The drawing under review shows one solid part. Ordinate dimensions are in mm from its lowest x, y, z. A direction names the side the tool comes from. Coordinates: 2 decimals unless noted, no trailing zeros. Loops run counter-clockwise (first coordinate to the right, second up) from the corner with the lowest first, then second, coordinate; pieces in that order, holes last. Notation, with made-up numbers: (40.5, -11) - (46.5, -11) arc R14 cw to (46.5, 6) - close; hole circle Ø7 at (77.25, 79.25). An arc over 180 degrees is marked (long way). Answer as a JSON object with one key per item and string values. Group by question number.
Item 1: We need section A-A (z = 3.5). Give the boundary of the cut face in (x, y).
Item 2: Clearance check with a flat-ended pin moving along its axis: pin 1 (1.5 mm diameter, centred on y = 3.5, z = 3, fed in from -X). State where the tip first meets the part, or that it passes through.
Item 3: We need section D-D (z = 6.25). Give the boundary of the cut face in (x, y).
Item 4: To check wall thickness, follow line 1 (X direction, y = 1.65, z = 3.5); line 2 (X direction, y = 2.3, z = 4.25); line 3 (Z direction, x = 24.5, y = 2.15). State the ranges of each line that lie inside material, in increasing order.
Item 5: Mouldability with a two-part tool opening along Z and no side actions: class the marked faces 3, 4 and 5 as released by +Z, released by -Z, zero draft, split by the parting line, or undercut.
Item 6: We need section B-B (y = 3.2). Give the boundary of the cut face in (x, z), then the cut area to 3 significant figures.
Item 7: Tool access review of the marked faces 1 and 2: name each direction out of +Z, -Z, +X, -X, +Y, -Y from which nothing blocks a thin tool from reaching the whole face with its end or side.
Item 8: We need section C-C (x = 28.5). Give the boundary of the cut face in (y, z), then the cut area to 3 significant figures.
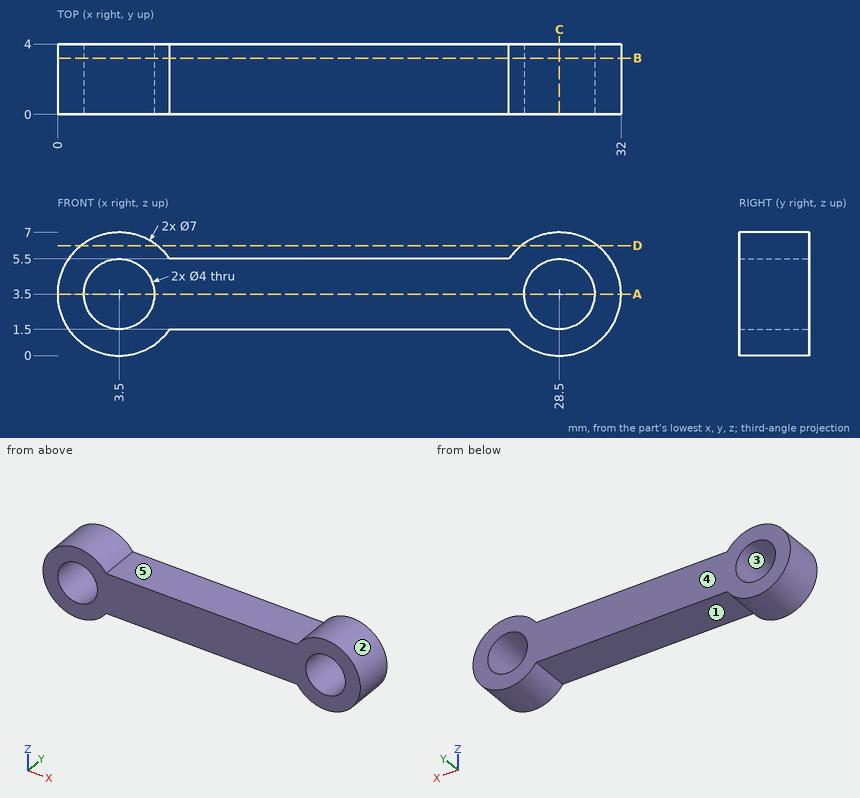
Check sheet entries:
{
 "1": {"outline": "(0, 0) - (1.5, 0) - (1.5, 4) - (0, 4) - close; (5.5, 0) - (26.5, 0) - (26.5, 4) - (5.5, 4) - close; (30.5, 0) - (32, 0) - (32, 4) - (30.5, 4) - close"},
 "2": {"pin 1": "stops at x = 0"},
 "3": {"outline": "(1.33, 0) - (5.67, 0) - (5.67, 4) - (1.33, 4) - close; (26.33, 0) - (30.67, 0) - (30.67, 4) - (26.33, 4) - close"},
 "4": {"line 1": "x = 0 to 1.5, 5.5 to 26.5, 30.5 to 32", "line 2": "x = 0.08 to 1.65, 5.35 to 26.65, 30.35 to 31.92", "line 3": "z = 1.5 to 5.5"},
 "5": {"face 3": "undercut", "face 4": "zero draft", "face 5": "released by +Z"},
 "6": {"outline": "(6.37, 1.5) - (25.63, 1.5) arc R3.5 ccw (long way) to (25.63, 5.5) - (6.37, 5.5) arc R3.5 ccw (long way) to start; hole circle Ø4 at (3.5, 3.5); hole circle Ø4 at (28.5, 3.5)", "area": "125 mm2"},
 "7": {"face 1": "-Z, +Y, -Y", "face 2": "+Y, -Y"},
 "8": {"outline": "(0, 0) - (4, 0) - (4, 1.5) - (0, 1.5) - close; (0, 5.5) - (4, 5.5) - (4, 7) - (0, 7) - close", "area": "12.0 mm2"}
}
